from build123d import *

# Parameters (mm, degrees)
SLOTTED_BASE_PLATE_DEPTH = 10
UPRIGHT_WEB_SKETCH_R     = 14
UPRIGHT_WEB_DEPTH        = 10
CLEVIS_ARM_DEPTH         = 40
CLEVIS_EAR_1_SKETCH_R    = 20
CLEVIS_EAR_1_DEPTH       = 10
CLEVIS_START             = -10
CLEVIS_EAR_2_SKETCH_R    = 20
CLEVIS_EAR_2_DEPTH       = 10
CLEVIS_PIN_HOLE_SKETCH_R = 9
CLEVIS_PIN_HOLE_18_DEPTH = 141.841641644


with BuildPart() as part:
    # Base Plate Sketch → Slotted Base Plate (new body)
    with BuildSketch(Plane(origin=(0, 0, 0), x_dir=(1, 0, 0), z_dir=(0, 1, 0))):
        with BuildLine():
            Line((0, 0), (-70, 0))
            Line((-70, 0), (-70, -14))
            ThreePointArc((-70, -14), (-65.313708499, -25.313708499), (-54, -30))
            Line((-54, -30), (-16, -30))
            ThreePointArc((-16, -30), (-4.686291501, -25.313708499), (0, -14))
            Line((0, -14), (0, 0))
        make_face()
        with BuildLine():
            Line((-54, -6), (-16, -6))
            ThreePointArc((-16, -6), (-8, -14), (-16, -22))
            Line((-16, -22), (-54, -22))
            ThreePointArc((-54, -22), (-62, -14), (-54, -6))
        make_face(mode=Mode.SUBTRACT)
    extrude(amount=SLOTTED_BASE_PLATE_DEPTH)

    # Upright Web Sketch → Upright Web (add)
    with BuildSketch(Plane(origin=(0, 0, 0), x_dir=(-1, 0, 0), z_dir=(0, 0, -1))):
        with BuildLine():
            Line((70, 0), (70, 34))
            ThreePointArc((70, 34), (49.281681362, 78.430577701), (1.928405695, 91.118849675))
            Line((1.928405695, 91.118849675), (-50.610518395, 81.85481982))
            Line((-50.610518395, 81.85481982), (-43.664591288, 42.4625097))
            Line((-43.664591288, 42.4625097), (-23.472963553, 46.022838454))
            ThreePointArc((-23.472963553, 46.022838454), (-7.144247806, 41.647572256), (0, 26.326683394))
            Line((0, 26.326683394), (0, 0))
            Line((0, 0), (70, 0))
        make_face()
        with Locations((35, 34)):
            Circle(UPRIGHT_WEB_SKETCH_R, mode=Mode.SUBTRACT)
    extrude(amount=UPRIGHT_WEB_DEPTH)

    # Clevis Arm Sketch → Clevis Arm (add)
    with BuildSketch(Plane(origin=(15.524092466, 88.041503368, 0), x_dir=(0.9848077530122072, -0.17364817766693494, 0), z_dir=(0.17364817766693494, 0.9848077530122072, 0))):
        Polygon((35.627690604, 27.5), (45.627690604, 27.5), (65.627690604, 27.5), (65.627690604, 17.5), (45.627690604, 17.5), (45.627690604, -7.5), (65.627690604, -7.5), (65.627690604, -17.5), (35.627690604, -17.5), align=None)
    extrude(amount=-CLEVIS_ARM_DEPTH)

    # Clevis Ear 1 Sketch → Clevis Ear 1 (add)
    with BuildSketch(Plane.XY.offset(17.5)):
        with Locations((76.681787432, 56.94921943)):
            Circle(CLEVIS_EAR_1_SKETCH_R)
    extrude(amount=-CLEVIS_EAR_1_DEPTH)

    # Clevis Ear 2 Sketch → Clevis Ear 2 (add)
    with BuildSketch(Plane(origin=(0, 0, -27.5), x_dir=(-1, 0, 0), z_dir=(0, 0, -1)).offset(CLEVIS_START)):
        with Locations((-76.681787432, 56.94921943)):
            Circle(CLEVIS_EAR_2_SKETCH_R)
    extrude(amount=CLEVIS_EAR_2_DEPTH)

    # Clevis Pin Hole Sketch → Clevis Pin Hole Ø18 (cut, through all)
    with BuildSketch(Plane.XY.offset(17.5)):
        with Locations((76.681787432, 56.94921943)):
            Circle(CLEVIS_PIN_HOLE_SKETCH_R)
    extrude(amount=-CLEVIS_PIN_HOLE_18_DEPTH, mode=Mode.SUBTRACT)


solid = part.part
The listing builds one solid part. Answer for the finished solid, in the listing's coordinates (mm). A direction names the side the tool comes from. Give positions to 0.01 mm unless a question says otherwise; leave off trailing zeros. Loops run counter-clockwise (first coordinate to the right, second up) from the corner with the lowest first, then second, coordinate; pieces in that order, holes last. Notation, with made-up numbers: (68, 36) - (110, 36) arc R14 ccw to (110, 53) - close; hole circle Ø8 at (89, 9.25). An arc over 180 degrees is marked (long way). Write each question's results on one line, items separated by ' | '.
1. Find section D-D, the plane y = 74. Write down the section's boundary in (x, z).
Resolved:
outline: (-54, -10) - (49.23, -10) - (49.23, -27.5) - (87.14, -27.5) - (87.14, -17.5) - (59.38, -17.5) - (59.38, 7.5) - (87.14, 7.5) - (87.14, 17.5) - (49.23, 17.5) - (49.23, 0) - (-54, 0) - close
2. Consider probe 1 along Z at (x, y) = (-3, 14.5); probe 2 along Y at (x, z) = (-31, 23.5); probe 3 along X at (y, z) = (24, -0.5). Determine where each line is inside the solid, lowest interval first. Write a range as from..to.
Resolved:
probe 1: z = -10..0 | probe 2: y = 0..10 | probe 3: x = -70..-44.8, -25.2..0
3. Find section A-A, the plane z = 3. Write down the section's boundary in (x, y), then the cut area to 3 significant figures.
Resolved:
outline: (-70, 0) - (0, 0) - (0, 10) - (-70, 10) - close; (43.66, 42.46) - (53.51, 40.73) - (60.46, 80.12) - (50.61, 81.85) - close | area: 1,100 mm^2
4. Find section B-B, the plane x = -35. Write down the section's boundary in (y, z).
Resolved:
outline: (0, -10) - (20, -10) - (20, 0) - (10, 0) - (10, 6) - (0, 6) - close; (0, 22) - (10, 22) - (10, 30) - (0, 30) - close; (48, -10) - (87.24, -10) - (87.24, 0) - (48, 0) - close
5. Find section C-C, the plane z = -23.5. Write down the section's boundary in (x, y).
Resolved:
outline: (43.66, 42.46) - (73.21, 37.25) arc R20 ccw to (80.15, 76.65) - (50.61, 81.85) - close; hole circle Ø18 at (76.68, 56.95)
6. Flat-ended cylindrical pins translate along their axes: P1, Ø1.5, axis at y = 68, z = -6, coming from the +X side; P2, Ø6, axis at x = -7, y = 80, coming from the -Z side; P3, Ø13.5, axis at x = 65.5, y = 58, coming from the +Z side. Find the tip coordinate at first contact, or state that the pin passes through.
Resolved:
P1: stops at x = 58.45 | P2: stops at z = -10 | P3: stops at z = 17.5
7. For a pull along Y with two mould halves and no side action, classify faces 1 (the face through (84.996, 53.502, -22.43)), 2 (the face through (47.186, 62.434, 8.872)), 3 (the face through (-9, 52, 0)) as +Y half, -Y half, draft (parallel to the pull), parting line (faces both ways), or undercut.
Resolved:
face 1: undercut | face 2: +Y half | face 3: draft
8. Which of the six approach directions +Z, -Z, +X, -X, +Y, -Y give full straight-line access (tool end or side, diameter ignored) to faces 4 (the face through (-8, 5, 14)), 5 (the face through (-35, 10, 5)), 6 (the face through (0, 10.4, -0.5))?
Resolved:
face 4: +Y, -Y | face 5: +Z, +X, -X, +Y | face 6: +Z, -Z, +X, -Y
